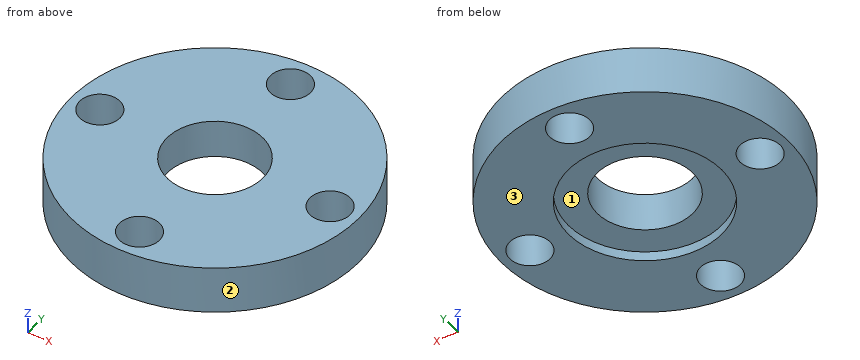
from build123d import *

# Parameters (mm, degrees)
SKETCH1_R           = 15
BOSS_EXTRUDE1_DEPTH = 5
SKETCH2_R           = 2.1
CUT_EXTRUDE1_DEPTH  = 22.794494718
CIRPATTERN1_COUNT   = 4
SKETCH3_R           = 8
CUT_EXTRUDE2_DEPTH  = 1
SKETCH4_R           = 5
CUT_EXTRUDE3_DEPTH  = 22.794494718


with BuildPart() as part:
    # Sketch1 → Boss-Extrude1 (new body)
    with BuildSketch(Plane.XY):
        Circle(SKETCH1_R)
    extrude(amount=BOSS_EXTRUDE1_DEPTH)

    # Sketch2 → Cut-Extrude1 (cut, through all)
    with BuildSketch(Plane.XY.offset(5)):
        with Locations((0, 12)):
            Circle(SKETCH2_R)
    cut_extrude1 = extrude(amount=-CUT_EXTRUDE1_DEPTH, mode=Mode.SUBTRACT)

    # CirPattern1: Cut-Extrude1 ×4 about axis
    cirpattern1_axis = Axis((0, 0, 0), (0, 0, 1))
    for i in range(1, CIRPATTERN1_COUNT):
        add(cut_extrude1.rotate(cirpattern1_axis, i * 360 / CIRPATTERN1_COUNT), mode=Mode.SUBTRACT)

    # Sketch3 → Cut-Extrude2 (cut)
    with BuildSketch(Plane(origin=(0, 0, 0), x_dir=(-1, 0, 0), z_dir=(0, 0, -1))):
        Circle(SKETCH3_R)
    extrude(amount=-CUT_EXTRUDE2_DEPTH, mode=Mode.SUBTRACT)

    # Sketch4 → Cut-Extrude3 (cut, through all)
    with BuildSketch(Plane.XY.offset(5)):
        Circle(SKETCH4_R)
    extrude(amount=-CUT_EXTRUDE3_DEPTH, mode=Mode.SUBTRACT)


solid = part.part
Model file for the job. Use its own axes, mm. Face numbers are marked on the shaded views. Coordinates: 2 decimals unless noted, no trailing zeros. Loops run counter-clockwise (first coordinate to the right, second up) from the corner with the lowest first, then second, coordinate; pieces in that order, holes last. Notation, with made-up numbers: (34.25, 3) -> (59.25, 3) arc R7 ccw to (59.25, 8) -> close; hole circle Ø10 at (54, -21.75). An arc over 180 degrees is marked (long way). Use one line per item in the form item = value. Start each with the question number.
(1) Pull direction Y, two halves, no side cores. Call the marked faces 1, 2 and 3: pulls with the +Y half, pulls with the -Y half, needs draft (parallel to the pull), parting line crosses it, or undercut.
(2) Cut at B-B on y = 0. Give the cut face in (x, z).
(3) Flat gauge pins, fed straight in: pin 1 (3 mm diameter, centred on y = 8.5, z = 4, fed in from -X); pin 2 (4 mm diameter, centred on x = 12, y = 0, fed in from +Z); pin 3 (1 mm diameter, centred on x = 4, z = 3, fed in from -Y); pin 4 (1 mm diameter, centred on x = 2.5, z = 2, fed in from +Y). Where does each tip first touch, or does it go through?
(4) Cut at A-A on x = 12. Give the cut face in (y, z).
(5) Probe probe 1 along Y at (x, z) = (0, 0.5); probe 2 along Y at (x, z) = (0, 3.4); probe 3 along X at (y, z) = (0.75, 0.6). List the from-to ranges inside material, lowest first. Write a range as from..to.
Values:
q1.face_1 = undercut
q1.face_2 = parting line crosses it
q1.face_3 = needs draft
q2.outline = (-15, 0) -> (-14.1, 0) -> (-14.1, 5) -> (-15, 5) -> close; (-9.9, 0) -> (-8, 0) -> (-8, 1) -> (-5, 1) -> (-5, 5) -> (-9.9, 5) -> close; (5, 1) -> (8, 1) -> (8, 0) -> (9.9, 0) -> (9.9, 5) -> (5, 5) -> close; (14.1, 0) -> (15, 0) -> (15, 5) -> (14.1, 5) -> close
q3.pin_1 = -13.27
q3.pin_2 = through
q3.pin_3 = -14.59
q3.pin_4 = 14.87
q4.outline = (-9, 0) -> (-2.1, 0) -> (-2.1, 5) -> (-9, 5) -> close; (2.1, 0) -> (9, 0) -> (9, 5) -> (2.1, 5) -> close
q5.probe_1 = -15..-14.1, -9.9..-8, 8..9.9, 14.1..15
q5.probe_2 = -15..-14.1, -9.9..-5, 5..9.9, 14.1..15
q5.probe_3 = -14.98..-13.96, -10.04..-7.96, 7.96..10.04, 13.96..14.98
